```python
from build123d import *

# Parameters (mm, degrees)
SKETCH_1_W          = 200
SKETCH_1_H          = 200
EXTRUDE_1_DEPTH     = 10
SKETCH_2_R          = 7
SKETCH_2_R_2        = 15
CUT_EXTRUDE_1_DEPTH = 284.019433962
CHAMFER_1_SIZE      = 5


with BuildPart() as part:
    # 草图1 → 凸台-拉伸1 (new body)
    with BuildSketch(Plane.XY):
        with Locations((100, -100)):
            Rectangle(SKETCH_1_W, SKETCH_1_H)
    extrude(amount=EXTRUDE_1_DEPTH)

    # 草图2 → 切除-拉伸1 (cut, through all)
    with BuildSketch(Plane.XY.offset(10)):
        with Locations((40, -55)):
            Circle(SKETCH_2_R)
        with Locations((40, -145)):
            Circle(SKETCH_2_R)
        with Locations((160, -145)):
            Circle(SKETCH_2_R)
        with Locations((160, -55)):
            Circle(SKETCH_2_R)
        with Locations((100, -100)):
            Circle(SKETCH_2_R_2)
    extrude(amount=-CUT_EXTRUDE_1_DEPTH, mode=Mode.SUBTRACT)

    # 倒角1
    chamfer_1_edges = [part.edges().sort_by_distance(p)[0] for p in [
        (0, 0, 5),
        (200, 0, 5),
        (200, -200, 5),
        (0, -200, 5),
    ]]
    chamfer(chamfer_1_edges, length=CHAMFER_1_SIZE)


solid = part.part
```
The model under review builds one solid part; all positions refer to its coordinate system, in mm. Round coordinates to 2 decimals unless told otherwise and drop trailing zeros. Order: outer loops, then holes, each group sorted by start corner. A loop starts at its lowest first (then second) coordinate and runs counter-clockwise, first axis right, second up.
Item 1: To check wall thickness, follow probe 1 along Y at (x, z) = (40, 6.5); probe 2 along X at (y, z) = (-145.5, 6.75); probe 3 along Y at (x, z) = (100, 7). State the ranges of each line that lie inside material, in increasing order.
Working result:
probe 1: y = -200 to -152, -138 to -62, -48 to 0
probe 2: x = 0 to 33.02, 46.98 to 153.02, 166.98 to 200
probe 3: y = -200 to -115, -85 to 0
Item 2: For pin 1 (11 mm diameter, centred on x = 40, y = -145, fed in from -Z), flat-tipped, find the tip position at first contact; note if it passes through.
Working result:
pin 1: passes through
Item 3: Add section B-B, the plane x = 160. State the section outline as (y, z) points, and give its area (3 significant figures).
Working result:
outline: (-200, 0) - (-152, 0) - (-152, 10) - (-200, 10) - close; (-138, 0) - (-62, 0) - (-62, 10) - (-138, 10) - close; (-48, 0) - (0, 0) - (0, 10) - (-48, 10) - close
area: 1,720 mm2
Item 4: Add section D-D, the plane z = 1.75. State the section outline as (x, y) points.
Working result:
outline: (0, -195) - (5, -200) - (195, -200) - (200, -195) - (200, -5) - (195, 0) - (5, 0) - (0, -5) - close; hole circle Ø14 at (40, -145); hole circle Ø14 at (40, -55); hole circle Ø30 at (100, -100); hole circle Ø14 at (160, -145); hole circle Ø14 at (160, -55)
Item 5: Add section A-A, the plane y = -100. State the section outline as (x, z) points, and give its area (3 significant figures).
Working result:
outline: (0, 0) - (85, 0) - (85, 10) - (0, 10) - close; (115, 0) - (200, 0) - (200, 10) - (115, 10) - close
area: 1,700 mm2
Item 6: Add section C-C, the plane y = -145. State the section outline as (x, z) points.
Working result:
outline: (0, 0) - (33, 0) - (33, 10) - (0, 10) - close; (47, 0) - (153, 0) - (153, 10) - (47, 10) - close; (167, 0) - (200, 0) - (200, 10) - (167, 10) - close
Item 7: Draft analysis for pull direction X (two halves, no side actions). For faces 1 (the flat face through (76, -99, 0)), 2 (the cylindrical face through (166.466, -147.681, 5.07)), 3 (the flat face through (0, -101, 5)), state which applies: released by +X, released by -X, zero draft, split by the parting line, or undercut.
Working result:
face 1: zero draft
face 2: undercut
face 3: released by -X
